Verification items for the finished model (mm, model axes). Face numbers are marked on the shaded views. Give positions to 0.01 mm unless a question says otherwise; leave off trailing zeros. Order: outer loops, then holes, each group sorted by start corner. A loop starts at its lowest first (then second) coordinate and runs counter-clockwise, first axis right, second up.
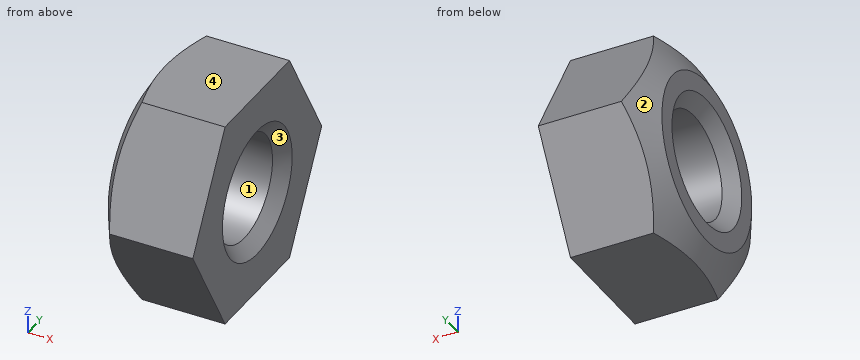
from build123d import *

# Parameters (mm, degrees)
SKETCH3_W          = 16
SKETCH3_H          = 16
CUT_EXTRUDE1_DEPTH = 4


with BuildPart() as part:
    # Sketch1 → Revolve1 (revolve)
    with BuildSketch(Plane.XY, mode=Mode.PRIVATE) as revolve1_sk:
        Polygon((-4, 0), (-4, 3.22), (-2.937675505, 5.06), (0, 5.06), (0, 0), align=None)
    revolve(revolve1_sk.sketch.rotate(Axis((0, 0, 0), (-1, 0, 0)), 270), axis=Axis((0, 0, 0), (-1, 0, 0)))

    # Sketch2 → Cut-Revolve1 (revolve, cut)
    with BuildSketch(Plane.XY, mode=Mode.PRIVATE) as cut_revolve1_sk:
        Polygon((-4, 0), (-4, 2.5), (-3.508532, 2.008532), (-0.491468, 2.008532), (0, 2.5), (0, 0), align=None)
    revolve(cut_revolve1_sk.sketch.rotate(Axis((0, 0, 0), (-1, 0, 0)), 270), axis=Axis((0, 0, 0), (-1, 0, 0)), mode=Mode.SUBTRACT)

    # Sketch3 → Cut-Extrude1 (cut)
    with BuildSketch(Plane(origin=(0, 0, 0), x_dir=(0, 0, -1), z_dir=(1, 0, 0))):
        Rectangle(SKETCH3_W, SKETCH3_H)
        Polygon((-4, 2.309401077), (-4, -2.309401077), (0, -4.618802154), (4, -2.309401077), (4, 2.309401077), (0, 4.618802154), align=None, mode=Mode.SUBTRACT)
    extrude(amount=-CUT_EXTRUDE1_DEPTH, mode=Mode.SUBTRACT)


solid = part.part
(1) Section check B-B, the plane x = -2.75. Enter the section's corners in (y, z).
Solved:
outline: (-4.62, 0) - (-2.31, -4) - (2.31, -4) - (4.62, 0) - (2.31, 4) - (-2.31, 4) - close; hole circle Ø4.02 at (0, 0)
(2) Scan lines: line 1 (Y direction, x = -2.9, z = 0.5); line 2 (Z direction, x = -2.7, y = 0.75); line 3 (Y direction, x = -2.75, z = 1). Record each from-to range of solid material in increasing order.
Solved:
line 1: y = -4.33 to -1.95, 1.95 to 4.33
line 2: z = -4 to -1.86, 1.86 to 4
line 3: y = -4.04 to -1.74, 1.74 to 4.04
(3) Go/stop test with flat-tipped pins: pin 1 (2 mm diameter, centred on x = -3.5, z = -2, fed in from -Y); pin 2 (2 mm diameter, centred on x = -3.5, z = -2.5, fed in from +Y). Record where each tip stops, or that it passes through.
Solved:
pin 1: stops at y = -4.04
pin 2: stops at y = 3.75
(4) Section check A-A, the plane y = 0. Enter the section's corners in (x, z).
Solved:
outline: (-4, -3.22) - (-3.55, -4) - (0, -4) - (0, -2.5) - (-0.49, -2.01) - (-3.51, -2.01) - (-4, -2.5) - close; (-4, 2.5) - (-3.51, 2.01) - (-0.49, 2.01) - (0, 2.5) - (0, 4) - (-3.55, 4) - (-4, 3.22) - close
(5) Release check for a two-part mould opening along Z. For the marked faces 1, 2, 3 and 4 record: pulls with the +Z half, pulls with the -Z half, needs draft (parallel to the pull), parting line crosses it, or undercut.
Solved:
face 1: undercut
face 2: parting line crosses it
face 3: undercut
face 4: pulls with the +Z half
